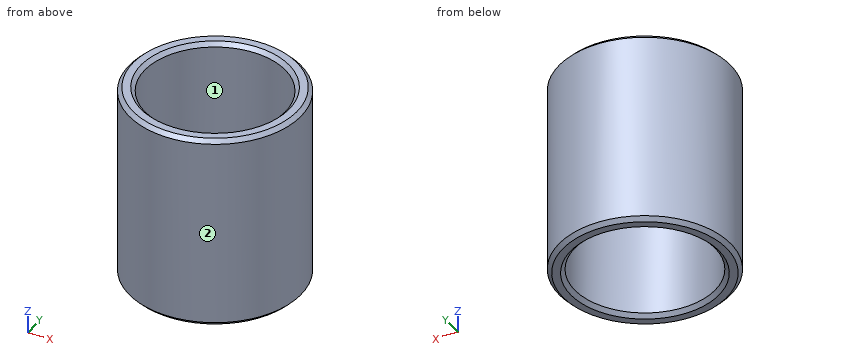
```python
from build123d import *

# Parameters (mm, degrees)
SKETCH_1_R      = 11
SKETCH_1_R_2    = 9
EXTRUDE_1_DEPTH = 25
CHAMFER_1_SIZE  = 0.5


with BuildPart() as part:
    # 草图1 → 凸台-拉伸1 (new body)
    with BuildSketch(Plane.XY):
        Circle(SKETCH_1_R)
        Circle(SKETCH_1_R_2, mode=Mode.SUBTRACT)
    extrude(amount=EXTRUDE_1_DEPTH)

    # 倒角1
    chamfer_1_edges = [part.edges().sort_by_distance(p)[0] for p in [
        (-11, 0, 0),
        (-11, 0, 25),
        (-9, 0, 0),
        (-9, 0, 25),
    ]]
    chamfer(chamfer_1_edges, length=CHAMFER_1_SIZE)


solid = part.part
```
Part model, mm, in its own coordinate system. Face numbers are marked on the shaded views. Round coordinates to 2 decimals unless told otherwise and drop trailing zeros. Loops run counter-clockwise (first coordinate to the right, second up) from the corner with the lowest first, then second, coordinate; pieces in that order, holes last. Notation, with made-up numbers: (-20, 13.25) -> (26, 13.25) arc R24 ccw to (26, 44.25) -> close; hole circle Ø11 at (60, -19). An arc over 180 degrees is marked (long way). Use a Markdown table: item, result.
1) Cut at C-C, the plane z = 4.25. List the corners of the cut face in (x, y), and give its area (3 significant figures).
The answers:
| item | result |
|---|---|
| outline | circle Ø22 at (0, 0); hole circle Ø18 at (0, 0) |
| area | 126 mm2 |
2) Drop flat-ended pins along their axis: pin 1 Ø5 at (y, z) = (9, 4) entering from +X; pin 2 Ø4 at (x, z) = (2.5, 7.5) entering from +Y; pin 3 Ø2 at (x, y) = (7, -4.5) entering from +Z. Give the stop position or say it passes through.
The answers:
| item | result |
|---|---|
| pin 1 | stops at x = 8.87 |
| pin 2 | stops at y = 10.99 |
| pin 3 | stops at z = 24.82 |
3) Pull direction X, two halves, no side cores. Call the marked faces 1 and 2: pulls with the +X half, pulls with the -X half, needs draft (parallel to the pull), parting line crosses it, or undercut.
The answers:
| item | result |
|---|---|
| face 1 | undercut |
| face 2 | parting line crosses it |
4) Cut at A-A, the plane x = 0. List the corners of the cut face in (y, z), and give its area (3 significant figures).
The answers:
| item | result |
|---|---|
| outline | (-11, 0.5) -> (-10.5, 0) -> (-9.5, 0) -> (-9, 0.5) -> (-9, 24.5) -> (-9.5, 25) -> (-10.5, 25) -> (-11, 24.5) -> close; (9, 0.5) -> (9.5, 0) -> (10.5, 0) -> (11, 0.5) -> (11, 24.5) -> (10.5, 25) -> (9.5, 25) -> (9, 24.5) -> close |
| area | 99.0 mm2 |
5) Probe line 1 (Y direction, x = 0, z = 7); line 2 (X direction, y = -7.5, z = 10); line 3 (Y direction, x = -5, z = 14.5). List the from-to ranges inside material, lowest first. Write a range as [from, to].
The answers:
| item | result |
|---|---|
| line 1 | y = [-11, -9], [9, 11] |
| line 2 | x = [-8.05, -4.97], [4.97, 8.05] |
| line 3 | y = [-9.8, -7.48], [7.48, 9.8] |
